Check sheet for the modelled part. Datum: model origin and axes. Units: mm. Face numbers are marked on the shaded views. A direction names the side the tool comes from. Coordinates: 2 decimals unless noted, no trailing zeros. Write each loop counter-clockwise with the first axis right and the second up, starting at its lowest first coordinate (ties: lowest second). Pieces come first, ordered by that corner, then holes. Notation, with made-up numbers: M 8.5,41.5 L 26.5,41.5 A10 ccw 26.5,58.5 Z; hole C 63,48 d5. An arc over 180 degrees is marked long. Answer as CSV lines item,"result".
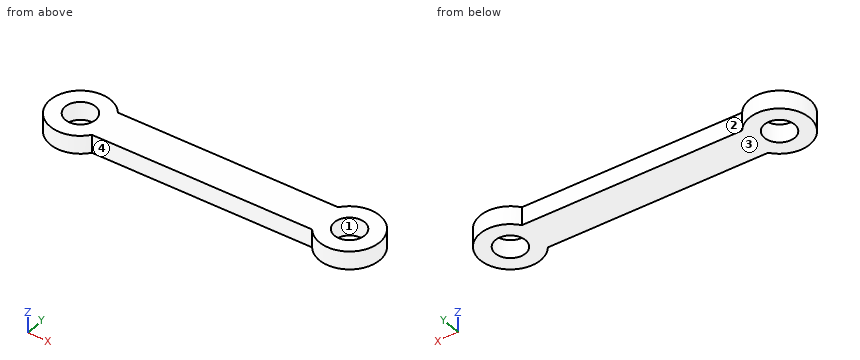
from build123d import *

# Parameters (mm, degrees)
SKETCH1_R           = 2.5
BOSS_EXTRUDE1_DEPTH = 3


with BuildPart() as part:
    # Sketch1 → Boss-Extrude1 (new body)
    with BuildSketch(Plane.XY):
        with BuildLine():
            Line((4, 3), (40, 3))
            ThreePointArc((40, 3), (49, 0), (40, -3))
            Line((40, -3), (4, -3))
            ThreePointArc((4, -3), (-5, 0), (4, 3))
        make_face()
        Circle(SKETCH1_R, mode=Mode.SUBTRACT)
        with Locations((44, 0)):
            Circle(SKETCH1_R, mode=Mode.SUBTRACT)
    extrude(amount=BOSS_EXTRUDE1_DEPTH)


solid = part.part
1) Thickness scan on line 1 along Y through (x, z) = (44, 0.9); line 2 along X through (y, z) = (0.25, 2.4); line 3 along X through (y, z) = (-0.5, 2.5). Record the ranges inside material, lowest first.
Answer key:
line 1,"y = -5 to -2.5, 2.5 to 5"
line 2,"x = -4.99 to -2.49, 2.49 to 41.51, 46.49 to 48.99"
line 3,"x = -4.97 to -2.45, 2.45 to 41.55, 46.45 to 48.97"
2) Section check A-A, the plane y = 0. Record the boundary of the cut face in (x, z).
Answer key:
outline,"M -5,0 L -2.5,0 L -2.5,3 L -5,3 Z; M 2.5,0 L 41.5,0 L 41.5,3 L 2.5,3 Z; M 46.5,0 L 49,0 L 49,3 L 46.5,3 Z"
3) Tool access check on the marked faces 1 and 2. Record the directions out of +Z, -Z, +X, -X, +Y, -Y that give a thin tool (end or side, any length) a straight path to the whole face; none if there is none.
Answer key:
face 1,"+Z, -Z"
face 2,"+Z, -Z, +Y"
4) Section check B-B, the plane x = 44. Record the boundary of the cut face in (y, z).
Answer key:
outline,"M -5,0 L -2.5,0 L -2.5,3 L -5,3 Z; M 2.5,0 L 5,0 L 5,3 L 2.5,3 Z"
5) Depth check by flat-ended pin: P1, Ø6, axis at x = 30.5, y = -3, coming from the -Z side; P2, Ø1, axis at y = 2, z = 1.5, coming from the +X side; P3, Ø1.5, axis at x = 14, z = 2, coming from the +Y side. Enter the tip coordinate at first touch or a pass-through.
Answer key:
P1,"stops at z = 0"
P2,"stops at x = 48.77"
P3,"stops at y = 3"
6) Mould release check, pull along X, two halves, no side actions. Record for the marked faces 3 and 4: pulls with the +X half, pulls with the -X half, needs draft (parallel to the pull), parting line crosses it, or undercut.
Answer key:
face 3,"needs draft"
face 4,"undercut"
7) Section check D-D, the plane y = 3.75. Record the boundary of the cut face in (x, z), plus the area to 3 significant figures.
Answer key:
outline,"M -3.31,0 L 3.31,0 L 3.31,3 L -3.31,3 Z; M 40.69,0 L 47.31,0 L 47.31,3 L 40.69,3 Z"
area,"39.7 mm2"
8) Section check C-C, the plane z = 0.8. Record the boundary of the cut face in (x, y), plus the area to 3 significant figures.
Answer key:
outline,"M 4,-3 L 40,-3 A5 ccw long 40,3 L 4,3 A5 ccw long Z; hole C 0,0 d5; hole C 44,0 d5"
area,"326 mm2"
